```python
from build123d import *

# Parameters (mm, degrees)
SKETCH1_W           = 500
SKETCH1_H           = 500
BOSS_EXTRUDE1_DEPTH = 600
SHELL1_T            = -10


with BuildPart() as part:
    # Sketch1 → Boss-Extrude1 (new body)
    with BuildSketch(Plane.XY):
        with Locations((250, 250)):
            Rectangle(SKETCH1_W, SKETCH1_H)
    extrude(amount=BOSS_EXTRUDE1_DEPTH)

    # Shell1
    shell1_openings = [part.faces().sort_by_distance(p)[0] for p in [
        (250, 250, 600),
    ]]
    offset(amount=SHELL1_T, openings=shell1_openings, kind=Kind.INTERSECTION)


solid = part.part
```
Verification items for the finished model (mm, model axes). A direction names the side the tool comes from. Coordinates: 2 decimals unless noted, no trailing zeros. Write each loop counter-clockwise with the first axis right and the second up, starting at its lowest first coordinate (ties: lowest second). Pieces come first, ordered by that corner, then holes. Notation, with made-up numbers: M 59.5,-38 L 109.5,-38 A27 ccw 109.5,-11 Z; hole C 74,22 d3. An arc over 180 degrees is marked long. Answer as a JSON object with one key per item and string values. Group by question number.
(1) Tool access check on faces 5 (the face through (0, 247, 296)), 6 (the face through (247, 490, 301)). Record the directions out of +Z, -Z, +X, -X, +Y, -Y that give a thin tool (end or side, any length) a straight path to the whole face; none if there is none.
(2) Material ranges on line 1 (Y direction, x = 458.5, z = 375.5); line 2 (Z direction, x = 316, y = 417.5), recorded low to high.
(3) Release check for a two-part mould opening along Y. For faces 1 (the face through (500, 247, 296)), 2 (the face through (247, 500, 296)), 3 (the face through (10, 247, 301)), 4 (the face through (490, 247, 301)) record: +Y half, -Y half, draft (parallel to the pull), parting line (faces both ways), or undercut.
(4) Cross-section at A-A, the plane z = 336.5. Record the cut outline in (x, y).
(5) Cross-section at B-B, the plane y = 204. Record the cut outline in (x, z), and give its area (3 significant figures).
(6) Gauge pin test, flat ends, axial feed: pin 1 (5 mm diameter, centred on x = 412.5, y = 109, fed in from +Z); pin 2 (5 mm diameter, centred on x = 158.5, y = 220.5, fed in from -Z). Record the tip position at first contact, or that the pin passes through.
Reply:
{
 "1": {"face 5": "+Z, -Z, -X, +Y, -Y", "face 6": "+Z"},
 "2": {"line 1": "0 to 10, 490 to 500", "line 2": "0 to 10"},
 "3": {"face 1": "draft", "face 2": "+Y half", "face 3": "undercut", "face 4": "undercut"},
 "4": {"outline": "M 0,0 L 500,0 L 500,500 L 0,500 Z; hole M 10,10 L 490,10 L 490,490 L 10,490 Z"},
 "5": {"outline": "M 0,0 L 500,0 L 500,600 L 490,600 L 490,10 L 10,10 L 10,600 L 0,600 Z", "area": "16,800 mm²"},
 "6": {"pin 1": "z = 10", "pin 2": "z = 0"}
}
